```python
from build123d import *

# Parameters (mm, degrees)
SKETCH1_W           = 60
SKETCH1_H           = 60
BOSS_EXTRUDE1_DEPTH = 35
SHELL1_T            = -5


with BuildPart() as part:
    # Sketch1 → Boss-Extrude1 (new body)
    with BuildSketch(Plane.XY):
        with Locations((-88, 0)):
            Rectangle(SKETCH1_W, SKETCH1_H)
    extrude(amount=BOSS_EXTRUDE1_DEPTH)

    # Shell1
    shell1_openings = [part.faces().sort_by_distance(p)[0] for p in [
        (-88, 0, 35),
    ]]
    offset(amount=SHELL1_T, openings=shell1_openings, kind=Kind.INTERSECTION)


solid = part.part
```
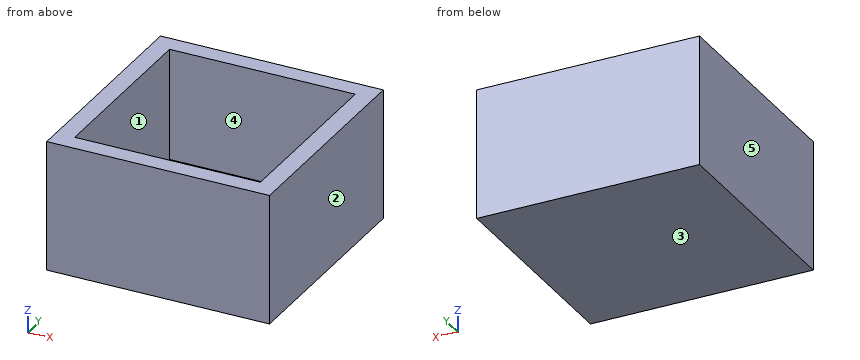
The listing builds one solid part. Answer for the finished solid, in the listing's coordinates (mm). Face numbers are marked on the shaded views. A direction names the side the tool comes from. Coordinates: 2 decimals unless noted, no trailing zeros. Write each loop counter-clockwise with the first axis right and the second up, starting at its lowest first coordinate (ties: lowest second). Pieces come first, ordered by that corner, then holes. Notation, with made-up numbers: M 78,-5.75 L 96,-5.75 A13 cw 96,5.25 Z; hole C -34,86.5 d9. An arc over 180 degrees is marked long. Use a Markdown table: item, result. Add a question column.
1. Section B-B (x = -101) is taken. Give the vertices of the cut face in (y, z), plus the area to 3 significant figures.
2. Straight lines are drawn through the part: line 1 along Y through (x, z) = (-97.5, 15.5); line 2 along X through (y, z) = (24.5, 8); line 3 along Z through (x, y) = (-98.5, -18). For each, find the intervals that lie inside material, in ascending order. Write a range as [from, to].
3. Given P1, Ø2, axis at x = -95.5, y = -7, coming from the +Z side, flat-ended and moving along its own axis, determine where the tip first touches the part or whether it passes through.
4. Section A-A (z = 23.5) is taken. Give the vertices of the cut face in (x, y).
5. Which of the six approach directions +Z, -Z, +X, -X, +Y, -Y give full straight-line access (tool end or side, diameter ignored) to the marked faces 4 and 5?
6. For a pull along X with two mould halves and no side action, classify the marked faces 1, 2 and 3 as +X half, -X half, draft (parallel to the pull), parting line (faces both ways), or undercut.
7. Section C-C (y = 9) is taken. Give the vertices of the cut face in (x, z).
Data:
| question | item | result |
|---|---|---|
| 1 | outline | M -30,0 L 30,0 L 30,35 L 25,35 L 25,5 L -25,5 L -25,35 L -30,35 Z |
| 1 | area | 600 mm2 |
| 2 | line 1 | y = [-30, -25], [25, 30] |
| 2 | line 2 | x = [-118, -113], [-63, -58] |
| 2 | line 3 | z = [0, 5] |
| 3 | P1 | stops at z = 5 |
| 4 | outline | M -118,-30 L -58,-30 L -58,30 L -118,30 Z; hole M -113,-25 L -63,-25 L -63,25 L -113,25 Z |
| 5 | face 4 | +Z |
| 5 | face 5 | +Z, -Z, -X, +Y, -Y |
| 6 | face 1 | undercut |
| 6 | face 2 | +X half |
| 6 | face 3 | draft |
| 7 | outline | M -118,0 L -58,0 L -58,35 L -63,35 L -63,5 L -113,5 L -113,35 L -118,35 Z |
